The model under review builds one solid part; all positions refer to its coordinate system, in mm. Round coordinates to 2 decimals unless told otherwise and drop trailing zeros. Loops run counter-clockwise (first coordinate to the right, second up) from the corner with the lowest first, then second, coordinate; pieces in that order, holes last. Notation, with made-up numbers: (34.5, 77) -> (92.5, 77) arc R27 cw to (92.5, 94) -> close; hole circle Ø10 at (-25.5, -27.5). An arc over 180 degrees is marked (long way). Use CSV: the item, a comma, the result in double quotes. Start each with the question number.
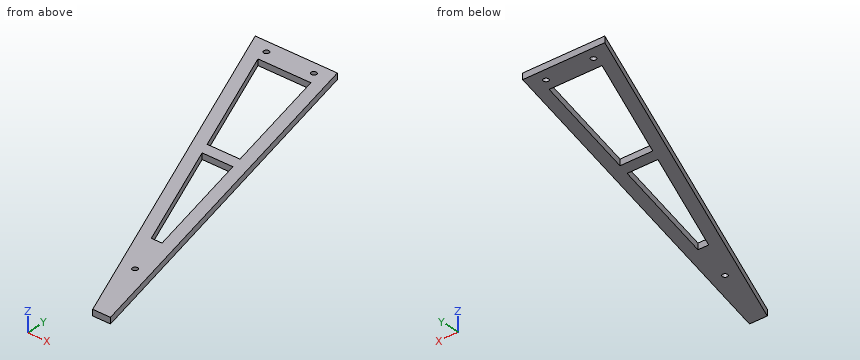
```python
from build123d import *

# Parameters (mm, degrees)
EXTRUDE_1_DEPTH     = 2.5
SKETCH_3_R          = 2.2
CUT_EXTRUDE_1_DEPTH = 10
CUT_EXTRUDE_2_DEPTH = 10
SKETCH_5_R          = 2.2
CUT_EXTRUDE_3_DEPTH = 10


with BuildPart() as part:
    # 草图1 → 凸台-拉伸1 (new, symmetric)
    with BuildSketch(Plane.XY):
        Polygon((255, -663), (171.307692308, -343), (102.153846154, -343), (240, -663), align=None)
    extrude(amount=EXTRUDE_1_DEPTH, both=True)

    # 草图3 → 切除-拉伸1 (cut)
    with BuildSketch(Plane.XY.offset(2.5)):
        with Locations((120.192307692, -353)):
            Circle(SKETCH_3_R)
        with Locations((160.192307692, -353)):
            Circle(SKETCH_3_R)
    extrude(amount=-CUT_EXTRUDE_1_DEPTH, mode=Mode.SUBTRACT)

    # 草图4 → 切除-拉伸2 (cut)
    with BuildSketch(Plane.XY.offset(2.5)):
        Polygon((166.202106442, -363), (121.657582941, -363), (164.734506018, -463), (192.355952596, -463), align=None)
        Polygon((194.971337211, -473), (169.042198326, -473), (212.119121403, -573), (221.125183365, -573), align=None)
    extrude(amount=-CUT_EXTRUDE_2_DEPTH, mode=Mode.SUBTRACT)

    # 草图5 → 切除-拉伸3 (cut)
    with BuildSketch(Plane.XY.offset(2.5)):
        with Locations((228.461538462, -608)):
            Circle(SKETCH_5_R)
    extrude(amount=-CUT_EXTRUDE_3_DEPTH, mode=Mode.SUBTRACT)


solid = part.part
```
1. Take a section at A-A, the plane z = 1. Give the boundary of the cut face in (x, y).
2. Take a section at D-D, the plane x = 114. Give the boundary of the cut face in (y, z).
3. Clearance check with flat-ended pins moving along their axes: P1, Ø1.5, axis at x = 177.5, z = -0.5, coming from the -Y side; P2, Ø5, axis at x = 120.19, y = -353, coming from the -Z side; P3, Ø1.5, axis at y = -602.5, z = 0, coming from the +X side. State where each tip first meets the part, or that it passes through.
4. Take a section at B-B, the plane y = -517. Give the boundary of the cut face in (x, z).
5. Take a section at C-C, the plane x = 129.5. Give the boundary of the cut face in (y, z), then the cut area to 3 significant figures.
6. For line 1 along X through (y, z) = (-353, -0.1); line 2 along X through (y, z) = (-423, 1.1); line 3 along Y through (x, z) = (139, 2.2), list the stretches that pass through material, from the lowest coordinate up. Write a range as from..to.
Results:
1,outline,"(102.15, -343) -> (240, -663) -> (255, -663) -> (171.31, -343) -> close; hole circle Ø4.4 at (120.19, -353); hole (121.66, -363) -> (164.73, -463) -> (192.36, -463) -> (166.2, -363) -> close; hole circle Ø4.4 at (160.19, -353); hole (169.04, -473) -> (212.12, -573) -> (221.13, -573) -> (194.97, -473) -> close; hole circle Ø4.4 at (228.46, -608)"
2,outline,"(-370.5, -2.5) -> (-343, -2.5) -> (-343, 2.5) -> (-370.5, 2.5) -> close"
3,P1,"y = -519.65"
3,P2,"z = -2.5"
3,P3,"x = 239.37"
4,outline,"(177.11, -2.5) -> (188, -2.5) -> (188, 2.5) -> (177.11, 2.5) -> close; (206.48, -2.5) -> (216.82, -2.5) -> (216.82, 2.5) -> (206.48, 2.5) -> close"
5,outline,"(-406.48, -2.5) -> (-381.21, -2.5) -> (-381.21, 2.5) -> (-406.48, 2.5) -> close; (-363, -2.5) -> (-343, -2.5) -> (-343, 2.5) -> (-363, 2.5) -> close"
5,area,"226 mm²"
6,line 1,"106.46..117.99, 122.39..157.99, 162.39..173.92"
6,line 2,"136.62..147.5, 181.89..192.23"
6,line 3,"-428.54..-403.26, -363..-343"
